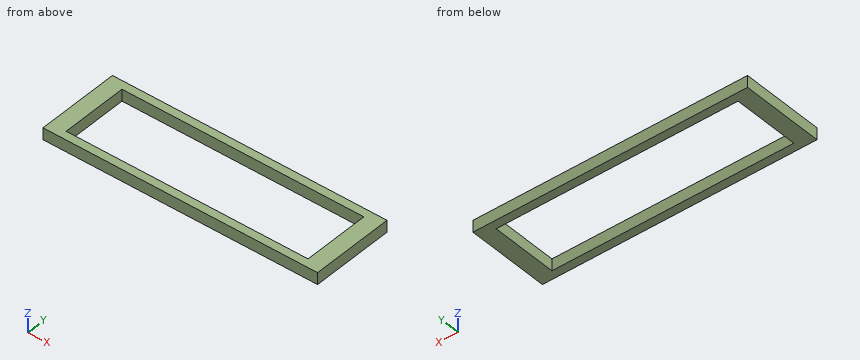
```python
from build123d import *

# Parameters (mm, degrees)
SKETCH_1_W      = 420
SKETCH_1_H      = 127
SKETCH_1_W_2    = 370
SKETCH_1_H_2    = 102
EXTRUDE_1_DEPTH = 9


with BuildPart() as part:
    # 草图1 → 凸台-拉伸1 (new, symmetric)
    with BuildSketch(Plane.XY):
        Rectangle(SKETCH_1_W, SKETCH_1_H)
        Rectangle(SKETCH_1_W_2, SKETCH_1_H_2, mode=Mode.SUBTRACT)
    extrude(amount=EXTRUDE_1_DEPTH, both=True)


solid = part.part
```
Check sheet for the modelled part. Datum: model origin and axes. Units: mm. Round coordinates to 2 decimals unless told otherwise and drop trailing zeros. Write each loop counter-clockwise with the first axis right and the second up, starting at its lowest first coordinate (ties: lowest second). Pieces come first, ordered by that corner, then holes. Notation, with made-up numbers: (-6.5, 27) -> (7.5, 27) arc R17 ccw to (7.5, 31) -> close; hole circle Ø3 at (-1.75, 81). An arc over 180 degrees is marked (long way). Put each result on its own line as item: value.
(1) Sectioned sample at A-A (x = 42.5). Enter the section's corners in (y, z).
Values found:
outline: (-63.5, -9) -> (-51, -9) -> (-51, 9) -> (-63.5, 9) -> close; (51, -9) -> (63.5, -9) -> (63.5, 9) -> (51, 9) -> close
(2) Material ranges on line 1 (Y direction, x = 14, z = 7.5); line 2 (X direction, y = 31.5, z = -3), recorded low to high.
Values found:
line 1: y = -63.5 to -51, 51 to 63.5
line 2: x = -210 to -185, 185 to 210
(3) Sectioned sample at B-B (z = -3.75). Enter the section's corners in (x, y), plus the area to 3 significant figures.
Values found:
outline: (-210, -63.5) -> (210, -63.5) -> (210, 63.5) -> (-210, 63.5) -> close; hole (-185, -51) -> (185, -51) -> (185, 51) -> (-185, 51) -> close
area: 15,600 mm^2
(4) Sectioned sample at C-C (y = -46). Enter the section's corners in (x, z), plus the area to 3 significant figures.
Values found:
outline: (-210, -9) -> (-185, -9) -> (-185, 9) -> (-210, 9) -> close; (185, -9) -> (210, -9) -> (210, 9) -> (185, 9) -> close
area: 900 mm^2
